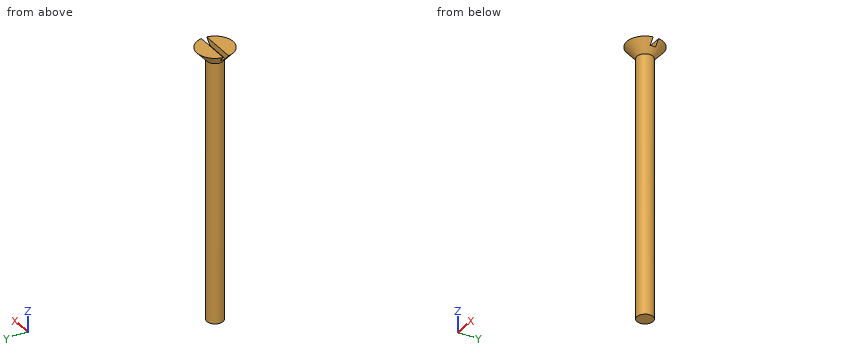
from build123d import *

# Parameters (mm, degrees)
SHANK_PROFILE_0_138_R       = 1.7526
SHANK_0_138_X_2_25_DEPTH    = 57.15
SCREWDRIVER_SLOT_DEPTH      = 60.952219472
SCREWDRIVER_SLOT_DEPTH_BACK = 60.952219472
SCREWDRIVER_SLOT_PROFILE_W  = 2.54
SCREWDRIVER_SLOT_PROFILE_H  = 1.168589104


with BuildPart() as part:
    # Shank Profile Ø0.138 → Shank Ø0.138 x 2.25 (new body)
    with BuildSketch(Plane.XY):
        Circle(SHANK_PROFILE_0_138_R)
    extrude(amount=SHANK_0_138_X_2_25_DEPTH)

    # Countersunk Head Profile → Countersunk Head 82° (revolve)
    with BuildSketch(Plane(origin=(0, 0, 0), x_dir=(0, 0, -1), z_dir=(1, 0, 0)), mode=Mode.PRIVATE) as countersunk_head_82_sk:
        Polygon((-57.15, 1.7526), (-59.69, 3.960588314), (-59.69, 0), (-57.15, 0), align=None)
    revolve(countersunk_head_82_sk.sketch.rotate(Axis((0, 0, 59.69), (0, 0, -1)), 180), axis=Axis((0, 0, 59.69), (0, 0, -1)))

    # Screwdriver Slot Profile → Screwdriver Slot (cut, two sides: drawn at the far end of the back side and taken through both)
    with BuildSketch(Plane(origin=(0, 0, 0), x_dir=(0, 0, -1), z_dir=(1, 0, 0)).offset(-SCREWDRIVER_SLOT_DEPTH_BACK)):
        with Locations((-59.69, 0)):
            Rectangle(SCREWDRIVER_SLOT_PROFILE_W, SCREWDRIVER_SLOT_PROFILE_H)
    extrude(amount=SCREWDRIVER_SLOT_DEPTH + SCREWDRIVER_SLOT_DEPTH_BACK, mode=Mode.SUBTRACT)


solid = part.part
Work out the finished part from the listing and answer in its coordinate system (mm). Give positions to 0.01 mm unless a question says otherwise; leave off trailing zeros. Loops run counter-clockwise (first coordinate to the right, second up) from the corner with the lowest first, then second, coordinate; pieces in that order, holes last. Notation, with made-up numbers: (87, -13) - (140, -13) arc R38 ccw to (140, 25) - close; hole circle Ø7 at (16.25, 68). An arc over 180 degrees is marked (long way). Answer in a Markdown table with one row per item.
(1) Flat-ended cylindrical pins translate along their axes: pin 1 Ø3 at (y, z) = (0.5, 12) entering from +X; pin 2 Ø3 at (x, z) = (-2, 21) entering from +Y; pin 3 Ø2 at (x, y) = (3, -1.5) entering from -Z. Find the tip coordinate at first contact, or state that the pin passes through.
Results list:
| item | result |
|---|---|
| pin 1 | stops at x = 1.75 |
| pin 2 | stops at y = 1.68 |
| pin 3 | stops at z = 57.84 |
(2) Section C-C (z = 21) is taken. Give the vertices of the cut face in (x, y).
Results list:
| item | result |
|---|---|
| outline | circle Ø3.51 at (0, 0) |
(3) Consider L1, parallel to Z at x = 1, y = -0.25; L2, parallel to Y at x = 1.5, z = 38; L3, parallel to X at y = 1.25, z = 47. Determine where each line is inside the solid, lowest interval first. Write a range as [from, to].
Results list:
| item | result |
|---|---|
| L1 | z = [0, 58.42] |
| L2 | y = [-0.91, 0.91] |
| L3 | x = [-1.23, 1.23] |
(4) Section B-B (x = 0) is taken. Give the vertices of the cut face in (y, z), and give its area (3 significant figures).
Results list:
| item | result |
|---|---|
| outline | (-3.96, 59.69) - (-1.75, 57.15) - (-1.75, 0) - (1.75, 0) - (1.75, 57.15) - (3.96, 59.69) - (0.58, 59.69) - (0.58, 58.42) - (-0.58, 58.42) - (-0.58, 59.69) - close |
| area | 213 mm² |
(5) Section A-A (y = 0) is taken. Give the vertices of the cut face in (x, z).
Results list:
| item | result |
|---|---|
| outline | (-2.86, 58.42) - (-1.75, 57.15) - (-1.75, 0) - (1.75, 0) - (1.75, 57.15) - (2.86, 58.42) - close |
